```python
from build123d import *

# Parameters (mm, degrees)
SKETCH1_W           = 550
SKETCH1_H           = 100
BOSS_EXTRUDE1_DEPTH = 10
SKETCH3_R           = 13
CUT_EXTRUDE2_DEPTH  = 5
SKETCH4_R           = 11
CUT_EXTRUDE3_DEPTH  = 280.55321497
SKETCH5_R           = 25
CUT_EXTRUDE4_DEPTH  = 280.687325419
SKETCH6_R           = 2.75
CUT_EXTRUDE5_DEPTH  = 280.687325419
SKETCH7_R           = 3.25
CUT_EXTRUDE6_DEPTH  = 280.687325419
FILLET1_R           = 1


with BuildPart() as part:
    # Sketch1 → Boss-Extrude1 (new body)
    with BuildSketch(Plane.XY):
        Rectangle(SKETCH1_W, SKETCH1_H)
    extrude(amount=BOSS_EXTRUDE1_DEPTH)

    # Sketch3 → Cut-Extrude2 (cut)
    with BuildSketch(Plane.XY.offset(10)):
        with Locations((225, 0)):
            Circle(SKETCH3_R)
        with Locations(Location((-225, 0, 0), (0, 0, 180))):
            Circle(SKETCH3_R)
    extrude(amount=-CUT_EXTRUDE2_DEPTH, mode=Mode.SUBTRACT)

    # Sketch4 → Cut-Extrude3 (cut, through all)
    with BuildSketch(Plane.XY.offset(5)):
        with Locations((225, 0)):
            Circle(SKETCH4_R)
        with Locations(Location((-225, 0, 0), (0, 0, 180))):
            Circle(SKETCH4_R)
    extrude(amount=-CUT_EXTRUDE3_DEPTH, mode=Mode.SUBTRACT)

    # Sketch5 → Cut-Extrude4 (cut, through all)
    with BuildSketch(Plane.XY.offset(10)):
        Circle(SKETCH5_R)
    extrude(amount=-CUT_EXTRUDE4_DEPTH, mode=Mode.SUBTRACT)

    # Sketch6 → Cut-Extrude5 (cut, through all)
    with BuildSketch(Plane.XY.offset(10)):
        with Locations((-24.748737342, 24.748737342)):
            Circle(SKETCH6_R)
        with Locations((24.748737342, 24.748737342)):
            Circle(SKETCH6_R)
        with Locations((24.748737342, -24.748737342)):
            Circle(SKETCH6_R)
        with Locations((-24.748737342, -24.748737342)):
            Circle(SKETCH6_R)
    extrude(amount=-CUT_EXTRUDE5_DEPTH, mode=Mode.SUBTRACT)

    # Sketch7 → Cut-Extrude6 (cut, through all)
    with BuildSketch(Plane.XY.offset(10)):
        with Locations((-120, -20)):
            Circle(SKETCH7_R)
        with Locations((120, -20)):
            Circle(SKETCH7_R)
        with Locations((120, 20)):
            Circle(SKETCH7_R)
        with Locations((-120, 20)):
            Circle(SKETCH7_R)
        with Locations((-120, 0)):
            Circle(SKETCH7_R)
        with Locations((120, 0)):
            Circle(SKETCH7_R)
    extrude(amount=-CUT_EXTRUDE6_DEPTH, mode=Mode.SUBTRACT)

    # Fillet1
    fillet1_edges = [part.edges().sort_by_distance(p)[0] for p in [
        (-275, 50, 5),
        (275, 50, 5),
        (275, -50, 5),
        (-275, -50, 5),
    ]]
    fillet(fillet1_edges, radius=FILLET1_R)

    # Sketch9 → M6 Tapped Hole1 (revolve, cut)
    with BuildSketch(Plane(origin=(-275, -35, 5), x_dir=(0, 0, 1), z_dir=(0, 1, 0))):
        Polygon((0, 0), (0, 19.502151548), (2.5, 18), (2.5, 0), align=None)
    m6_tapped_hole1 = revolve(axis=Axis((-281.35, -35, 5), (1, 0, 0)), mode=Mode.SUBTRACT)

    # Mirror1: M6 Tapped Hole1 across plane
    add(m6_tapped_hole1.mirror(Plane(origin=(0, 0, 0), x_dir=(0, 0, 1), z_dir=(1, 0, 0))), mode=Mode.SUBTRACT)


solid = part.part
```
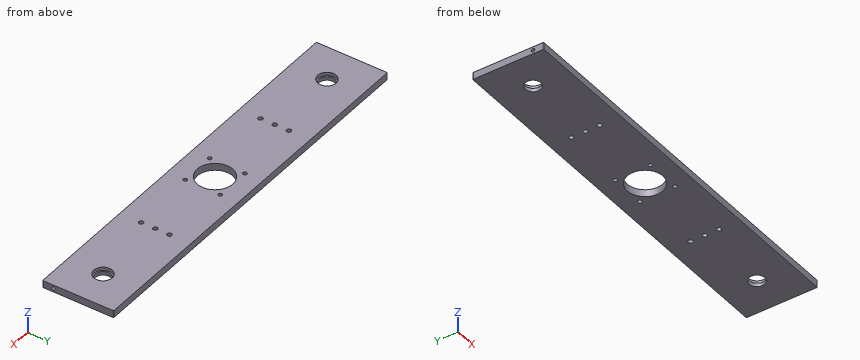
Source: CAD feature listing. Evaluate the final solid. Frame: model axes, mm. Give positions to 0.01 mm unless a question says otherwise; leave off trailing zeros. Loops run counter-clockwise (first coordinate to the right, second up) from the corner with the lowest first, then second, coordinate; pieces in that order, holes last. Notation, with made-up numbers: M 76.25,-39 L 91.25,-39 A16 cw 91.25,-27 Z; hole C 71.25,21 d3. An arc over 180 degrees is marked long. Put each result on its own line as item: value.
Q1. Section A-A (x = -225). Return the cut outline in (y, z), and give its area (3 significant figures).
Response values:
outline: M -50,0 L -11,0 L -11,5 L -13,5 L -13,10 L -50,10 Z; M 11,0 L 50,0 L 50,10 L 13,10 L 13,5 L 11,5 Z
area: 760 mm²
Q2. Line query: probe 1 along Y at (x, z) = (0, 6.25); probe 2 along Y at (x, z) = (-9, 2.5); probe 3 along X at (y, z) = (7.5, 7). Output: solid intervals per line, ascending. Write a range as [from, to].
Response values:
probe 1: y = [-50, -25], [25, 50]
probe 2: y = [-50, -23.32], [23.32, 50]
probe 3: x = [-275, -235.62], [-214.38, -23.85], [23.85, 214.38], [235.62, 275]
Q3. Pin query (flat end, axial travel): P1, Ø17.5, axis at x = -225, y = 0, coming from the -Z side; P2, Ø13, axis at x = 221.5, y = -4, coming from the +Z side; P3, Ø10.5, axis at x = 120, y = 20, coming from the -Z side. Return the tip coordinate at first contact, or that it passes through.
Response values:
P1: passes through
P2: stops at z = 5
P3: stops at z = 0
